For this review, use the dimensioned drawing (mm, ordinates from the lowest corner) and the shaded views. Coordinates: 2 decimals unless noted, no trailing zeros. Write each loop counter-clockwise with the first axis right and the second up, starting at its lowest first coordinate (ties: lowest second). Pieces come first, ordered by that corner, then holes.
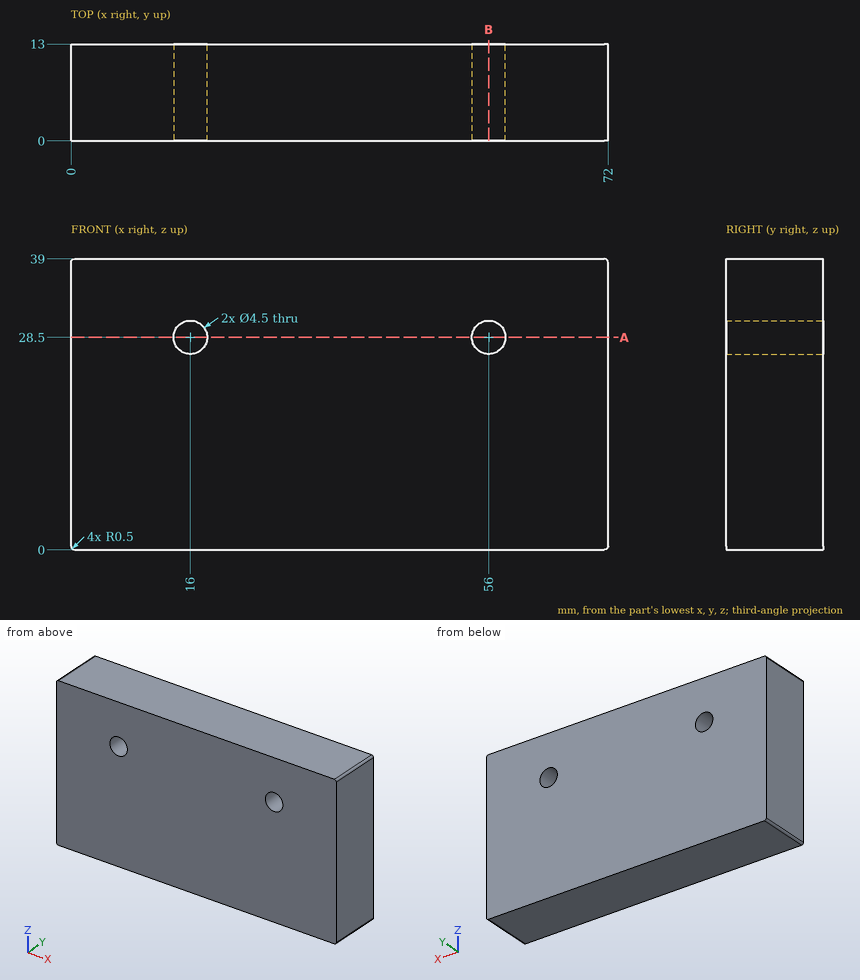
Item 1: Take a section at A-A, the plane z = 28.5. Write out the cut boundary in (x, y), plus the area to 3 significant figures.
Solved:
outline: (0, 0) - (13.75, 0) - (13.75, 13) - (0, 13) - close; (18.25, 0) - (53.75, 0) - (53.75, 13) - (18.25, 13) - close; (58.25, 0) - (72, 0) - (72, 13) - (58.25, 13) - close
area: 819 mm2
Item 2: To check wall thickness, follow line 1 along Z through (x, y) = (56, 5). State the ranges of the line that lie inside material, in increasing order.
Solved:
line 1: z = 0 to 26.25, 30.75 to 39
Item 3: Take a section at B-B, the plane x = 56. Write out the cut boundary in (y, z), plus the area to 4 significant figures.
Solved:
outline: (0, 0) - (13, 0) - (13, 26.25) - (0, 26.25) - close; (0, 30.75) - (13, 30.75) - (13, 39) - (0, 39) - close
area: 448.5 mm2
